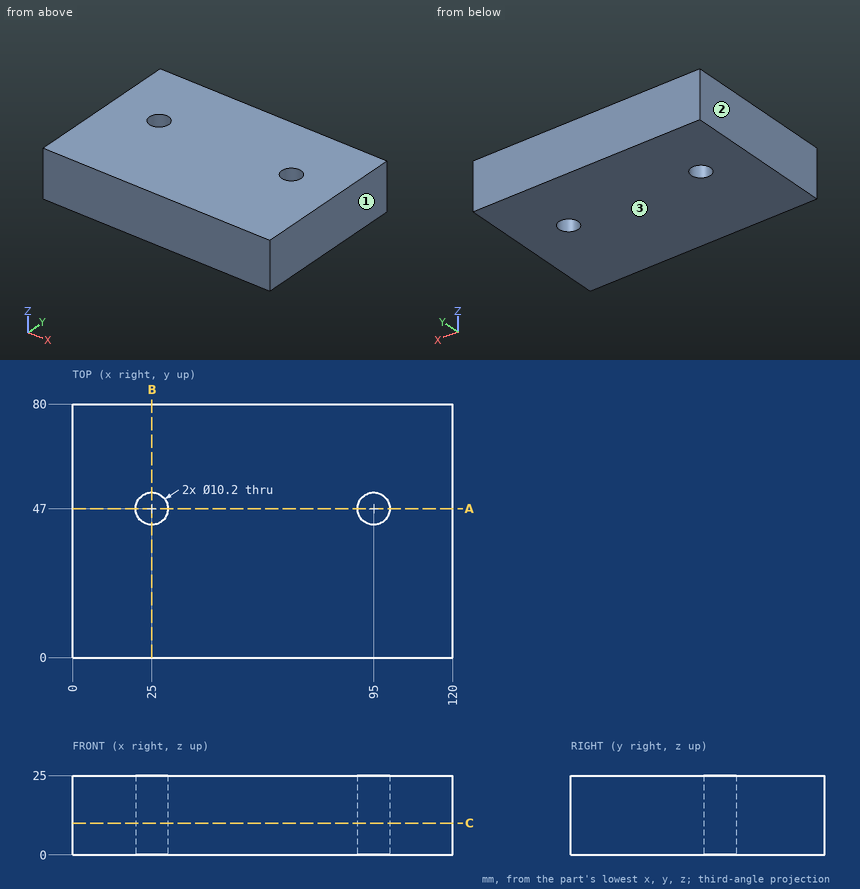
The figure shows three views and two pictorial views of one solid part (mm, origin at its lowest corner). Answer the questions. Give positions to 0.01 mm unless a question says otherwise; leave off trailing zeros. Order: outer loops, then holes, each group sorted by start corner. A loop starts at its lowest first (then second) coordinate and runs counter-clockwise, first axis right, second up. Notation, with made-up numbers: M 46.25,-12 L 76.25,-12 A26 cw 76.25,22 Z; hole C 23,2 d1. An arc over 180 degrees is marked long. Return JSON: item names as keys, results as strings.
1) Straight lines are drawn through the part: line 1 along X through (y, z) = (46, 11.75); line 2 along Y through (x, z) = (95, 14); line 3 along Y through (x, z) = (99.5, 8.5). For each, find the intervals that lie inside material, in ascending order. Write a range as [from, to].
Resolved:
{"line 1": "[0, 20], [30, 90], [100, 120]", "line 2": "[0, 41.9], [52.1, 80]", "line 3": "[0, 44.6], [49.4, 80]"}
2) Section B-B, the plane x = 25 is taken. Write down the section's boundary in (y, z).
Resolved:
{"outline": "M 0,0 L 41.9,0 L 41.9,25 L 0,25 Z; M 52.1,0 L 80,0 L 80,25 L 52.1,25 Z"}
3) Each of these flat-tipped pins is pushed along its axis until it touches: pin 1 (1 mm diameter, centred on x = 15.5, y = 11, fed in from -Z); pin 2 (9 mm diameter, centred on x = 95, y = 47, fed in from +Z). Where does it stop, or does it pass through?
Resolved:
{"pin 1": "z = 0", "pin 2": "through"}
4) Section C-C, the plane z = 10 is taken. Write down the section's boundary in (x, y).
Resolved:
{"outline": "M 0,0 L 120,0 L 120,80 L 0,80 Z; hole C 25,47 d10.2; hole C 95,47 d10.2"}
5) Section A-A, the plane y = 47 is taken. Write down the section's boundary in (x, z), plus the area to 3 significant figures.
Resolved:
{"outline": "M 0,0 L 19.9,0 L 19.9,25 L 0,25 Z; M 30.1,0 L 89.9,0 L 89.9,25 L 30.1,25 Z; M 100.1,0 L 120,0 L 120,25 L 100.1,25 Z", "area": "2,490 mm^2"}
6) For a pull along X with two mould halves and no side action, classify the marked faces 1, 2 and 3 as +X half, -X half, draft (parallel to the pull), parting line (faces both ways), or undercut.
Resolved:
{"face 1": "+X half", "face 2": "-X half", "face 3": "draft"}
